Design review of the part built by this model. Coordinates are the model's own, in mm. Coordinates: 2 decimals unless noted, no trailing zeros. Loops run counter-clockwise (first coordinate to the right, second up) from the corner with the lowest first, then second, coordinate; pieces in that order, holes last. Notation, with made-up numbers: (16, 74) -> (25, 74) arc R8 ccw to (25, 89) -> close; hole circle Ø9 at (38, 5). An arc over 180 degrees is marked (long way). Answer as a JSON object with one key per item and string values.
```python
from build123d import *

# Parameters (mm, degrees)
SKETCH1_R                   = 5
BOSS_EXTRUDE1_DEPTH         = 60
SKETCH2_R                   = 1.5
BOSS_EXTRUDE2_DEPTH         = 90
M4_TAPPED_HOLE1_D           = 3.3
M4_TAPPED_HOLE1_DEPTH       = 11.5
M4_TAPPED_HOLE1_CSINK_D     = 4.05
M4_TAPPED_HOLE1_CSINK_ANGLE = 90
M4_TAPPED_HOLE1_TIP         = 0.991420021


with BuildPart() as part:
    # Sketch1 → Boss-Extrude1 (new body)
    with BuildSketch(Plane(origin=(0, 0, 0), x_dir=(1, 0, 0), z_dir=(0, 1, 0))):
        with Locations(Location((0, 0, 0), (0, 0, 270))):
            Circle(SKETCH1_R)
    extrude(amount=BOSS_EXTRUDE1_DEPTH)

    # Sketch2 → Boss-Extrude2 (add)
    with BuildSketch(Plane(origin=(0, 60, 0), x_dir=(1, 0, 0), z_dir=(0, 1, 0))):
        with Locations(Location((0, 0, 0), (0, 0, 90))):
            Circle(SKETCH2_R)
    extrude(amount=BOSS_EXTRUDE2_DEPTH)

    # M4 Tapped Hole1
    with Locations(Plane(origin=(0, 0, 0), x_dir=(-1, 0, 0), z_dir=(0, -1, 0))):
        with Locations((0, 0)):
            CounterSinkHole(M4_TAPPED_HOLE1_D / 2, M4_TAPPED_HOLE1_CSINK_D / 2, depth=M4_TAPPED_HOLE1_DEPTH, counter_sink_angle=M4_TAPPED_HOLE1_CSINK_ANGLE)
            with Locations((0, 0, -(M4_TAPPED_HOLE1_DEPTH + M4_TAPPED_HOLE1_TIP / 2))):  # 118° drill point
                Cone(0, M4_TAPPED_HOLE1_D / 2, M4_TAPPED_HOLE1_TIP, mode=Mode.SUBTRACT)


solid = part.part
```
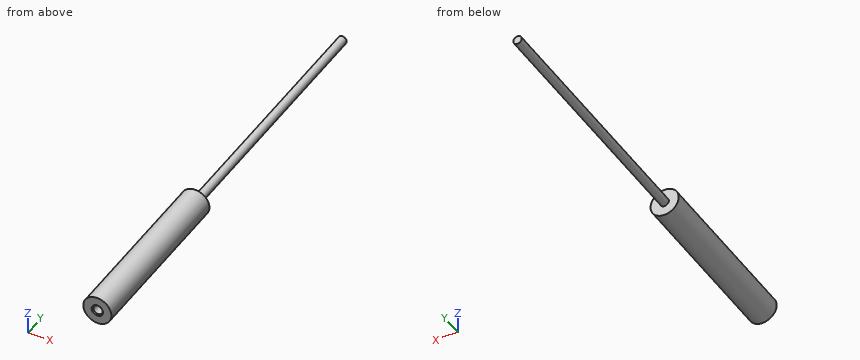
1) Clearance check with flat-ended pins moving along their axes: pin 1 Ø3 at (x, z) = (-3.5, -3) entering from -Y; pin 2 Ø3 at (y, z) = (132.5, -2.5) entering from +X; pin 3 Ø2 at (x, z) = (-3.5, 1.5) entering from +Y; pin 4 Ø2 at (x, y) = (1.5, 107.5) entering from +Z. State where each tip first meets the part, or that it passes through.
Completed:
{"pin 1": "y = 0", "pin 2": "x = 1.12", "pin 3": "y = 60", "pin 4": "z = 1.41"}
2) Add section C-C, the plane z = -3.25. Give the boundary of the cut face in (x, y), and give its area (3 significant figures).
Completed:
{"outline": "(-3.8, 0) -> (3.8, 0) -> (3.8, 60) -> (-3.8, 60) -> close", "area": "456 mm²"}
3) Add section B-B, the plane x = -3.75. Give the boundary of the cut face in (y, z).
Completed:
{"outline": "(0, -3.31) -> (60, -3.31) -> (60, 3.31) -> (0, 3.31) -> close"}
4) Add section A-A, the plane y = 137. Give the boundary of the cut face in (x, z), and give its area (3 significant figures).
Completed:
{"outline": "circle Ø3 at (0, 0)", "area": "7.07 mm²"}
5) Wall thickness on probe 1 along Y at (x, z) = (0.5, -2); probe 2 along X at (y, z) = (31.5, 1.5); probe 3 along X at (y, z) = (131, -0.5): over which ranges is each line inside the solid? List them lowest first.
Completed:
{"probe 1": "0 to 60", "probe 2": "-4.77 to 4.77", "probe 3": "-1.41 to 1.41"}
